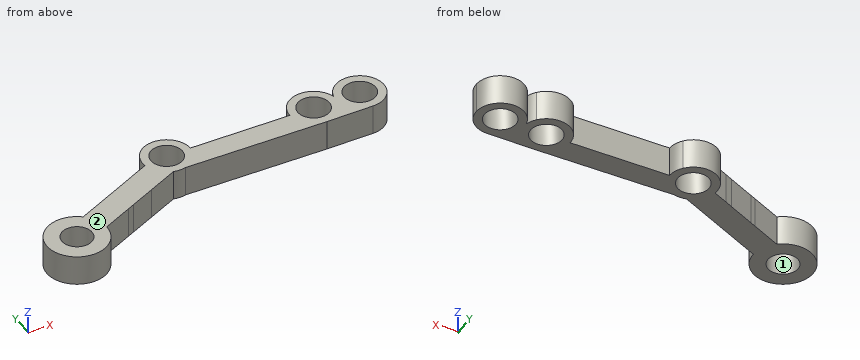
```python
from build123d import *

# Parameters (mm, degrees)
BOSS_EXTRUDE1_DEPTH  = 5
SKETCH3_R            = 2.5
CUT_EXTRUDE3_DEPTH   = 10
SKETCH2_R            = 1.5
CUT_EXTRUDE4_DEPTH   = 7
SKETCH5_R            = 4
BOSS_EXTRUDE2_DEPTH  = 5
SKETCH6_R            = 4
BOSS_EXTRUDE3_DEPTH  = 5
BOSS_EXTRUDE4_DEPTH  = 5
SKETCH9_R            = 4
BOSS_EXTRUDE5_DEPTH  = 5
SKETCH10_R           = 2.625
SKETCH10_R_2         = 2.5
CUT_EXTRUDE5_DEPTH   = 39.359537556
SKETCH11_R           = 4
BOSS_EXTRUDE6_DEPTH  = 5
SKETCH12_R           = 2.625
CUT_EXTRUDE6_DEPTH   = 39.359537556
SKETCH13_R           = 4
BOSS_EXTRUDE7_DEPTH  = 5
CUT_EXTRUDE7_DEPTH   = 39.359537556
CUT_EXTRUDE8_DEPTH   = 39.359537556
BOSS_EXTRUDE8_DEPTH  = 5
BOSS_EXTRUDE9_DEPTH  = 5
CUT_EXTRUDE9_DEPTH   = 10
CUT_EXTRUDE10_DEPTH  = 10
CUT_EXTRUDE11_DEPTH  = 10
CUT_EXTRUDE12_DEPTH  = 10
SKETCH30_R           = 2.5
BOSS_EXTRUDE16_DEPTH = 5


with BuildPart() as part:
    # Sketch1 → Boss-Extrude1 (new body)
    with BuildSketch(Plane.XY):
        with BuildLine():
            Line((0, 0), (34, 0))
            ThreePointArc((34, 0), (34.707106781, -0.292893219), (35, -1))
            Line((35, -1), (35, -4))
            ThreePointArc((35, -4), (34.707106781, -4.707106781), (34, -5))
            Line((34, -5), (0, -5))
            ThreePointArc((0, -5), (-4.600765263, -6.121207346), (-8.169848164, -9.233408201))
            ThreePointArc((-8.169848164, -9.233408201), (-8.772233245, -9.633451101), (-9.486832981, -9.522774425))
            Line((-9.486832981, -9.522774425), (-12.093386622, -8.017879978))
            ThreePointArc((-12.093386622, -8.017879978), (-12.567944885, -7.375988891), (-12.421485667, -6.591272758))
            ThreePointArc((-12.421485667, -6.591272758), (-7.030970465, -1.749888517), (0, 0))
        make_face()
    extrude(amount=BOSS_EXTRUDE1_DEPTH)

    # Sketch3 → Cut-Extrude3 (cut)
    with BuildSketch(Plane(origin=(0, 0, 0), x_dir=(-1, 0, 0), z_dir=(0, 0, -1))):
        with Locations((0, -2.5)):
            Circle(SKETCH3_R)
    extrude(amount=-CUT_EXTRUDE3_DEPTH, mode=Mode.SUBTRACT)


with BuildPart() as cut_extrude3_piece_1:
    # of the separate pieces the step leaves, piece 1, a body of its own (cut_extrude3_pieces)
    add(part.part.solids().sort_by_distance((34, 0, 0))[0])



with BuildPart() as cut_extrude3_piece_2:
    # of the separate pieces the step leaves, piece 2, a body of its own (cut_extrude3_pieces)
    add(part.part.solids().sort_by_distance((-12.421485667, -6.591272758, 0))[0])

    # Sketch2 → Cut-Extrude4 (cut)
    with BuildSketch(Plane.XY.offset(5)):
        with Locations((32.633829537, -2.570962999)):
            Circle(SKETCH2_R)
        with Locations((-9.587088302, -6.686632842)):
            Circle(SKETCH2_R)
        with Locations((24.694851026, -2.570962999)):
            Circle(SKETCH2_R)
    extrude(amount=-CUT_EXTRUDE4_DEPTH, mode=Mode.SUBTRACT)


with BuildPart() as cut_extrude3_piece_1_1:
    add(cut_extrude3_piece_1.part)

    add(cut_extrude3_piece_2.part)  # Boss-Extrude2 merges Cut-Extrude3 piece 2
    # Sketch5 → Boss-Extrude2 (add)
    with BuildSketch(Plane(origin=(0, 0, 0), x_dir=(-1, 0, 0), z_dir=(0, 0, -1))):
        with Locations((0, -2.5)):
            Circle(SKETCH5_R)
    extrude(amount=-BOSS_EXTRUDE2_DEPTH)

    # Sketch6 → Boss-Extrude3 (add, through all)
    with BuildSketch(Plane.XY.offset(5)):
        with Locations((16.69060283, -2.5)):
            Circle(SKETCH6_R)
    extrude(amount=-BOSS_EXTRUDE3_DEPTH)

    # Sketch7 → Boss-Extrude4 (add, through all)
    with BuildSketch(Plane.XY.offset(5)):
        with BuildLine():
            ThreePointArc((29.377501001, -5), (33.824764885, -6.274254628), (36.5, -2.5))
            ThreePointArc((36.5, -2.5), (33.824764885, 1.274254628), (29.377501001, 0))
            Line((29.377501001, 0), (34, 0))
            ThreePointArc((34, 0), (34.707106781, -0.292893219), (35, -1))
            Line((35, -1), (35, -2.5))
            Line((35, -2.5), (35, -4))
            ThreePointArc((35, -4), (34.707106781, -4.707106781), (34, -5))
            Line((34, -5), (29.377501001, -5))
        make_face()
    extrude(amount=-BOSS_EXTRUDE4_DEPTH)

    # Sketch9 → Boss-Extrude5 (add, through all)
    with BuildSketch(Plane.XY.offset(5)):
        with Locations((-9.587088302, -6.686632842)):
            Circle(SKETCH9_R)
    extrude(amount=-BOSS_EXTRUDE5_DEPTH)

    # Sketch10 → Cut-Extrude5 (cut, through all)
    with BuildSketch(Plane.XY.offset(5)):
        with Locations((0, -2.5)):
            Circle(SKETCH10_R)
        with Locations((-9.587088302, -6.686632842)):
            Circle(SKETCH10_R)
        with Locations((16.69060283, -2.5)):
            Circle(SKETCH10_R_2)
        with Locations((32.5, -2.5)):
            Circle(SKETCH10_R)
    extrude(amount=-CUT_EXTRUDE5_DEPTH, mode=Mode.SUBTRACT)

    # Sketch11 → Boss-Extrude6 (add, through all)
    with BuildSketch(Plane.XY.offset(5)):
        with Locations((24.694851026, -2.570962999)):
            Circle(SKETCH11_R)
    extrude(amount=-BOSS_EXTRUDE6_DEPTH)

    # Sketch12 → Cut-Extrude6 (cut, through all)
    with BuildSketch(Plane.XY.offset(5)):
        with Locations((24.694851026, -2.570962999)):
            Circle(SKETCH12_R)
    extrude(amount=-CUT_EXTRUDE6_DEPTH, mode=Mode.SUBTRACT)

    # Sketch13 → Boss-Extrude7 (add, through all)
    with BuildSketch(Plane.XY.offset(5)):
        with Locations((16.69060283, -2.5)):
            Circle(SKETCH13_R)
    extrude(amount=-BOSS_EXTRUDE7_DEPTH)

    # Sketch14 → Cut-Extrude7 (cut, through all)
    with BuildSketch(Plane.XY.offset(5)):
        Polygon((13.568103831, 0), (19.813101829, 0), (19.608152419, 3.101401215), (13.568103831, 2.844182656), (12.582024398, 1.287333479), align=None)
        Polygon((13.568103831, -5), (19.813101829, -5), (20.934648885, -7.644859521), (15.442425287, -9.366014099), (11.632678636, -7.644859521), align=None)
    extrude(amount=-CUT_EXTRUDE7_DEPTH, mode=Mode.SUBTRACT)

    # Sketch15 → Cut-Extrude8 (cut, through all)
    with BuildSketch(Plane.XY.offset(5)):
        Polygon((21.630515983, 0), (5.499420419, 2.191296742), (3.122498999, 0), align=None)
        with BuildLine():
            ThreePointArc((21.630515983, 0), (20.936038702, -1.202997388), (20.694851026, -2.570962999))
            Line((20.694851026, -2.570962999), (4, -2.5))
            ThreePointArc((4, -2.5), (3.774254628, -1.175235115), (3.122498999, 0))
            Line((3.122498999, 0), (21.630515983, 0))
        make_face()
        with BuildLine():
            Line((-7.607535591, 0.794757928), (-3.398220122, -0.39))
            ThreePointArc((-3.398220122, -0.39), (-6.16935857, -1.327435689), (-8.705842203, -2.784914591))
            Line((-8.705842203, -2.784914591), (-7.607535591, 0.794757928))
        make_face()
        with BuildLine():
            ThreePointArc((-3.398220122, -0.39), (-6.16935857, -1.327435689), (-8.705842203, -2.784914591))
            ThreePointArc((-8.705842203, -2.784914591), (-7.460532252, -3.29874864), (-6.456429886, -4.196858178))
            ThreePointArc((-6.456429886, -4.196858178), (-5.240156475, -3.557355191), (-3.961412583, -3.054265596))
            ThreePointArc((-3.961412583, -3.054265596), (-3.913518389, -1.672731107), (-3.398220122, -0.39))
        make_face()
        Polygon((28.45366335, 2.528160998), (29.377501001, 0), (27.75918607, 0), align=None)
        with BuildLine():
            Line((29.377501001, 0), (27.75918607, 0))
            ThreePointArc((27.75918607, 0), (28.271805382, -0.780600595), (28.589454783, -1.658788905))
            ThreePointArc((28.589454783, -1.658788905), (28.886992542, -0.783556844), (29.377501001, 0))
        make_face()
    extrude(amount=-CUT_EXTRUDE8_DEPTH, mode=Mode.SUBTRACT)

    # Sketch16 → Boss-Extrude8 (add, through all)
    with BuildSketch(Plane.XY.offset(5)):
        with BuildLine():
            Line((1.01271432, -6.369678243), (24.694851026, -6.570962999))
            Line((24.694851026, -6.570962999), (32.5, -6.5))
            Line((32.5, -6.5), (28.834380203, -3.557484395))
            Line((28.834380203, -3.557484395), (25.878705121, -5.379005085))
            Line((25.878705121, -5.379005085), (23.335449819, -5.379005085))
            Line((23.335449819, -5.379005085), (21.307719239, -4.244850693))
            Line((21.307719239, -4.244850693), (3.023775712, -3.866799229))
            Line((3.023775712, -3.866799229), (0.570007719, -5.379005085))
            Line((0.570007719, -5.379005085), (-2.853206137, -4.622902157))
            Line((-2.853206137, -4.622902157), (-6.221300997, -5.963266438))
            Line((-6.221300997, -5.963266438), (-6.565043066, -9.307175266))
            ThreePointArc((-6.565043066, -9.307175266), (-3.14075004, -6.897917977), (1.01271432, -6.369678243))
        make_face()
    extrude(amount=-BOSS_EXTRUDE8_DEPTH)

    # Sketch17 → Boss-Extrude9 (add)
    with BuildSketch(Plane(origin=(0, 0, 0), x_dir=(-1, 0, 0), z_dir=(0, 0, -1))):
        Polygon((3.961412583, -3.054265596), (13.495388719, -7.538212462), (11.30366334, -11.209638817), (1.01271432, -6.369678243), align=None)
    extrude(amount=-BOSS_EXTRUDE9_DEPTH)

    # Sketch18 → Cut-Extrude9 (cut)
    with BuildSketch(Plane(origin=(0, 0, 0), x_dir=(-1, 0, 0), z_dir=(0, 0, -1))):
        with BuildLine():
            Line((3.961412583, -3.054265596), (6.456429886, -4.196858178))
            ThreePointArc((6.456429886, -4.196858178), (5.240156475, -3.557355191), (3.961412583, -3.054265596))
        make_face()
    extrude(amount=-CUT_EXTRUDE9_DEPTH, mode=Mode.SUBTRACT)

    # Sketch19 → Cut-Extrude10 (cut)
    with BuildSketch(Plane(origin=(0, 0, 0), x_dir=(-1, 0, 0), z_dir=(0, 0, -1))):
        with BuildLine():
            Line((6.001656968, -8.71603966), (10.116735554, -10.651412003))
            ThreePointArc((10.116735554, -10.651412003), (7.658367525, -10.535986511), (6.001656968, -8.71603966))
        make_face()
    extrude(amount=-CUT_EXTRUDE10_DEPTH, mode=Mode.SUBTRACT)

    # Sketch20 → Cut-Extrude11 (cut)
    with BuildSketch(Plane(origin=(0, 0, 0), x_dir=(-1, 0, 0), z_dir=(0, 0, -1))):
        Polygon((6.456429886, -4.196858178), (7.733220064, -4.828193293), (12.200841034, -6.929370679), (14.105694097, -7.825246628), (14.33213787, -2.397708334), (7.630569976, -1.451472026), align=None)
    extrude(amount=-CUT_EXTRUDE11_DEPTH, mode=Mode.SUBTRACT)

    # Sketch21 → Cut-Extrude12 (cut)
    with BuildSketch(Plane(origin=(0, 0, 0), x_dir=(-1, 0, 0), z_dir=(0, 0, -1))):
        Polygon((11.30366334, -11.209638817), (13.114607064, -7.359126141), (14.222505477, -7.880184465), (12.35401945, -11.85304626), align=None)
    extrude(amount=-CUT_EXTRUDE12_DEPTH, mode=Mode.SUBTRACT)

    # Sketch30 → Boss-Extrude16 (add)
    with BuildSketch(Plane(origin=(0, 0, 0), x_dir=(-1, 0, 0), z_dir=(0, 0, -1))):
        with BuildLine():
            Line((13.114607064, -7.359126141), (11.30366334, -11.209638817))
            Line((11.30366334, -11.209638817), (16.258283795, -13.539858082))
            ThreePointArc((16.258283795, -13.539858082), (25.782858061, -15.668272182), (18.069227519, -9.689345407))
            Line((18.069227519, -9.689345407), (13.114607064, -7.359126141))
        make_face()
        with Locations((21.258283775, -13.540308948)):
            Circle(SKETCH30_R, mode=Mode.SUBTRACT)
    extrude(amount=-BOSS_EXTRUDE16_DEPTH)


solid = cut_extrude3_piece_1_1.part
```
Build history of the part. All positions in model axes, mm. Face numbers are marked on the shaded views. Give positions to 0.01 mm unless a question says otherwise; leave off trailing zeros. Loops run counter-clockwise (first coordinate to the right, second up) from the corner with the lowest first, then second, coordinate; pieces in that order, holes last. Notation, with made-up numbers: (34, -31.75) -> (49, -31.75) arc R28 ccw to (49, -11.75) -> close; hole circle Ø7 at (-16, 61). An arc over 180 degrees is marked (long way). One line per question, with ' | ' between items.
Q1. Pull direction X, two halves, no side cores. Call the marked faces 1 and 2: pulls with the +X half, pulls with the -X half, needs draft (parallel to the pull), parting line crosses it, or undercut.
Filled sheet:
face 1: undercut | face 2: needs draft
Q2. Cut at C-C, the plane z = 3.3. Count the separate pieces of the cut face and the enclosed holes in it, plus the area to 3 significant figures.
Filled sheet:
separate pieces: 1 | enclosed holes: 4 | area: 288 mm²
Q3. Cut at A-A, the plane x = 0. Write the cut outline in (y, z) (3 decimals).
Filled sheet:
outline: (-6.5, 0) -> (-5.125, 0) -> (-5.125, 5) -> (-6.5, 5) -> close; (0.125, 0) -> (1.5, 0) -> (1.5, 5) -> (0.125, 5) -> close
Q4. Cut at B-B, the plane y = -12.5. Write the cut outline in (x, z), plus the area to 3 significant figures.
Filled sheet:
outline: (-26.15, 0) -> (-23.53, 0) -> (-23.53, 5) -> (-26.15, 5) -> close; (-18.99, 0) -> (-14.05, 0) -> (-14.05, 5) -> (-18.99, 5) -> close | area: 37.8 mm²
Q5. Drill centre lines: line 1 along Y through (x, z) = (-21, 1.2); line 2 along X through (y, z) = (-1, 3.9); line 3 along X through (y, z) = (-3.25, 3.55). Where is each one in solid material? Low to high. Write a range as [from, to].
Filled sheet:
line 1: y = [-18.53, -16.03], [-11.05, -8.55] | line 2: x = [-3.71, -2.15], [2.15, 3.71], [21.02, 22.59], [26.8, 28.37], [28.79, 30.35], [34.65, 36.21] | line 3: x = [-4.39, -2.52], [2.52, 22.16], [27.23, 29.98], [35.02, 36.43]
